from build123d import *

# Parameters (mm, degrees)
SKETCH1_W          = 2
SKETCH1_H          = 20
SKETCH2_R          = 4
CUT_EXTRUDE1_DEPTH = 10
SCALE_1_SCALE      = 1.875


with BuildPart() as part:
    # Sketch1 → Revolve1 (revolve)
    with BuildSketch(Plane.XY, mode=Mode.PRIVATE) as revolve1_sk:
        with Locations((1, 55)):
            Rectangle(SKETCH1_W, SKETCH1_H)
    revolve(revolve1_sk.sketch.rotate(Axis((0, 0, 0), (1, 0, 0)), 90), axis=Axis((0, 0, 0), (1, 0, 0)))

    # Sketch2 → Cut-Extrude1 (cut)
    with BuildSketch(Plane(origin=(2, 0, 0), x_dir=(0, 0, -1), z_dir=(1, 0, 0))):
        with Locations((0, 55)):
            Circle(SKETCH2_R)
        with Locations((47.631397208, 27.5)):
            Circle(SKETCH2_R)
        with Locations((-47.631397208, 27.5)):
            Circle(SKETCH2_R)
        with Locations((47.631397208, -27.5)):
            Circle(SKETCH2_R)
        with Locations((-47.631397208, -27.5)):
            Circle(SKETCH2_R)
        with Locations((0, -55)):
            Circle(SKETCH2_R)
    extrude(amount=-CUT_EXTRUDE1_DEPTH, mode=Mode.SUBTRACT)


with BuildPart() as part_1:
    # Scale 1: scaled about (1, 0, 0)
    add(part.part.scale(SCALE_1_SCALE).moved(Location((-0.875, 0, 0))))


solid = part_1.part
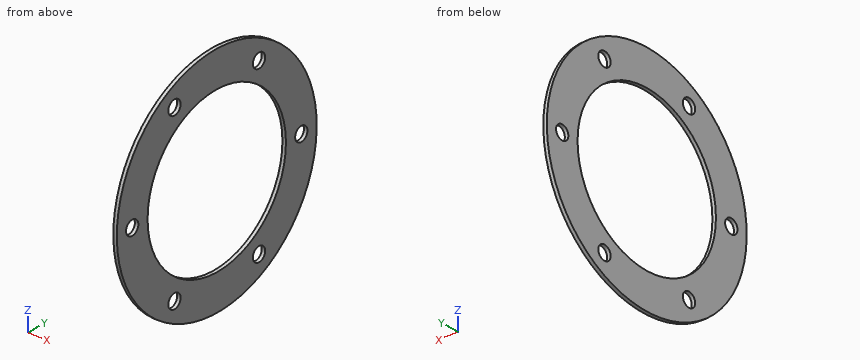
Check sheet for the modelled part. Datum: model origin and axes. Units: mm. Give positions to 0.01 mm unless a question says otherwise; leave off trailing zeros. Write each loop counter-clockwise with the first axis right and the second up, starting at its lowest first coordinate (ties: lowest second). Pieces come first, ordered by that corner, then holes. Notation, with made-up numbers: (-24.5, 40) -> (-2.5, 40) arc R30 cw to (-2.5, 63) -> close; hole circle Ø7 at (50.25, 65). An arc over 180 degrees is marked (long way). Use one line per item in the form item = value. Start each with the question number.
1. Thickness scan on line 1 along Y through (x, z) = (0, -1); line 2 along Y through (x, z) = (1.3, 0) (3 decimals); line 3 along Z through (x, y) = (2.05, 58). Record the ranges inside material, lowest first. Write a range as from..to.
2. Section check B-B (z = 0). Record the cut outline in (x, y) (3 decimals).
3. Go/stop test with flat-tipped pins: P1, Ø1.5, axis at x = 1, z = 91.5, coming from the +Y side; P2, Ø1, axis at x = 1.5, y = 58.5, coming from the -Z side. Record where each tip stops, or that it passes through.
4. Section check D-D (y = -48). Record the cut outline in (x, z) (3 decimals), and give its area (3 significant figures).
5. Section check A-A (y = 0). Record the cut outline in (x, z) (3 decimals), and give its area (3 significant figures).
6. Section check C-C (x = 0.6). Count the separate pieces of the cut face and the enclosed holes in it, and give its area (3 significant figures).
Conclusion:
q1.line_1 = -121.87..-110.56, -95.69..-84.37, 84.37..95.69, 110.56..121.87
q1.line_2 = -121.875..-110.625, -95.625..-84.375, 84.375..95.625, 110.625..121.875
q1.line_3 = -107.19..-93.16, -85.46..-61.28, 61.28..85.46, 93.16..107.19
q2.outline = (-0.875, -121.875) -> (2.875, -121.875) -> (2.875, -110.625) -> (-0.875, -110.625) -> close; (-0.875, -95.625) -> (2.875, -95.625) -> (2.875, -84.375) -> (-0.875, -84.375) -> close; (-0.875, 84.375) -> (2.875, 84.375) -> (2.875, 95.625) -> (-0.875, 95.625) -> close; (-0.875, 110.625) -> (2.875, 110.625) -> (2.875, 121.875) -> (-0.875, 121.875) -> close
q3.P1 = 81.35
q3.P2 = -107.19
q4.outline = (-0.875, -112.025) -> (2.875, -112.025) -> (2.875, -95.909) -> (-0.875, -95.909) -> close; (-0.875, -82.709) -> (2.875, -82.709) -> (2.875, -69.391) -> (-0.875, -69.391) -> close; (-0.875, 69.391) -> (2.875, 69.391) -> (2.875, 82.709) -> (-0.875, 82.709) -> close; (-0.875, 95.909) -> (2.875, 95.909) -> (2.875, 112.025) -> (-0.875, 112.025) -> close
q4.area = 221 mm²
q5.outline = (-0.875, -121.875) -> (2.875, -121.875) -> (2.875, -84.375) -> (-0.875, -84.375) -> close; (-0.875, 84.375) -> (2.875, 84.375) -> (2.875, 121.875) -> (-0.875, 121.875) -> close
q5.area = 281 mm²
q6.separate_pieces = 1
q6.enclosed_holes = 7
q6.area = 23,200 mm²
